For this review, take the finished solid that the model builds, in its own axes (mm). A direction names the side the tool comes from. Round coordinates to 2 decimals unless told otherwise and drop trailing zeros. Order: outer loops, then holes, each group sorted by start corner. A loop starts at its lowest first (then second) coordinate and runs counter-clockwise, first axis right, second up. Notation, with made-up numbers: (-39.75, 13) - (1.25, 13) arc R14 ccw to (1.25, 27) - close; hole circle Ø8 at (16.25, 3.5). An arc over 180 degrees is marked (long way). One line per question, with ' | ' between items.
```python
from build123d import *

# Parameters (mm, degrees)
BOSS_EXTRUDE1_DEPTH                               = 25
SKETCH2_W                                         = 18.5
SKETCH2_H                                         = 19
CUT_EXTRUDE1_DEPTH                                = 25
COUNTERBORE_FOR_PAN_HEAD_SCREW_OF_M61_D           = 6.6
COUNTERBORE_FOR_PAN_HEAD_SCREW_OF_M61_CBORE_D     = 13
COUNTERBORE_FOR_PAN_HEAD_SCREW_OF_M61_CBORE_DEPTH = 4.6
FILETE1_R                                         = 5
FILETE2_R                                         = 2


with BuildPart() as part:
    # Sketch1 → Boss-Extrude1 (new body)
    with BuildSketch(Plane(origin=(0, 0, 0), x_dir=(1, 0, 0), z_dir=(0, 1, 0))):
        Polygon((-52.5, 0), (52.5, 0), (65, -20), (65, -35), (45, -35), (45, -5), (-45, -5), (-45, -35), (-65, -35), (-65, -20), align=None)
    extrude(amount=BOSS_EXTRUDE1_DEPTH)

    # Sketch2 → Cut-Extrude1 (cut)
    with BuildSketch(Plane(origin=(0, 0, 0), x_dir=(-1, 0, 0), z_dir=(0, 0, -1))):
        with Locations((-58.75, 12.5)):
            Rectangle(SKETCH2_W, SKETCH2_H)
        with Locations((58.75, 12.5)):
            Rectangle(SKETCH2_W, SKETCH2_H)
    extrude(amount=-CUT_EXTRUDE1_DEPTH, mode=Mode.SUBTRACT)

    # Counterbore for pan head screw of M61 (through all)
    with Locations(Plane(origin=(0, 0, 25), x_dir=(-1, 0, 0), z_dir=(0, 0, -1))):
        with Locations((-57.25, 12.5), (57.25, 12.5)):
            CounterBoreHole(COUNTERBORE_FOR_PAN_HEAD_SCREW_OF_M61_D / 2, COUNTERBORE_FOR_PAN_HEAD_SCREW_OF_M61_CBORE_D / 2, COUNTERBORE_FOR_PAN_HEAD_SCREW_OF_M61_CBORE_DEPTH)

    # Filete1
    filete1_edges = [part.edges().sort_by_distance(p)[0] for p in [
        (-52.5, 23.5, 0),
        (52.5, 23.5, 0),
        (65, 23.5, 20),
        (-65, 23.5, 20),
        (52.5, 1.5, 0),
        (65, 1.5, 20),
        (-52.5, 1.5, 0),
        (-65, 1.5, 20),
    ]]
    fillet(filete1_edges, radius=FILETE1_R)

    # Filete2
    filete2_edges = [part.edges().sort_by_distance(p)[0] for p in [
        (45, 12.5, 5),
        (-45, 12.5, 5),
    ]]
    fillet(filete2_edges, radius=FILETE2_R)


solid = part.part
```
(1) Mouldability with a two-part tool opening along Y and no side actions: class faces 4 (the flat face through (-54, 14, 29.6)), 5 (the flat face through (59.03, 1.48, 10.45)) as released by +Y, released by -Y, zero draft, split by the parting line, or undercut.
Output values:
face 4: undercut | face 5: zero draft
(2) For faces 1 (the cylindrical face through (51.05, 14.45, 27.27)), 2 (the flat face through (56, 22, 15)), 3 (the flat face through (-55, 3, 15)), list the 3-axis set-ups (+Z, -Z, +X, -X, +Y, -Y) from which the entire face can be reached by the end or side of a thin tool; tool diameter is ignored.
Output values:
face 1: -Z | face 2: -Z, +X | face 3: -Z, -X
(3) For probe 1 along X at (y, z) = (10.5, 18); probe 2 along X at (y, z) = (12, 32); probe 3 along Y at (x, z) = (-57.25, 28.25), list the stretches that pass through material, from the lowest coordinate up. Write a range as [from, to].
Output values:
probe 1: [-49.5, -45], [45, 49.5] | probe 2: [-65, -60.51], [-53.99, -45], [45, 53.99], [60.51, 65] | probe 3: [0, 6], [19, 25]
(4) We need section A-A on z = 16. State the section outline as (x, y) points, plus the area to 3 significant figures.
Output values:
outline: (-62.5, 0) - (-45, 0) - (-45, 25) - (-62.5, 25) - (-62.5, 22) - (-49.5, 22) - (-49.5, 3) - (-62.5, 3) - close; (45, 0) - (62.5, 0) - (62.5, 3) - (49.5, 3) - (49.5, 22) - (62.5, 22) - (62.5, 25) - (45, 25) - close | area: 381 mm^2
(5) Insertion check: pin 1 (8 mm diameter, centred on x = 57, y = 12.5, fed in from -Z); pin 2 (4 mm diameter, centred on y = 21.5, z = 6.5, fed in from -X); pin 3 (6 mm diameter, centred on y = 21, z = 18, fed in from +X). Each pin has a flat end and moves straight along its axis. Give the tip position at first contact, or say it passes through.
Output values:
pin 1: z = 29.6 | pin 2: x = -57.77 | pin 3: x = 64.96
(6) We need section B-B on x = 57.25. State the section outline as (y, z) points, plus the area to 3 significant figures.
Output values:
outline: (0, 7.6) - (3, 7.6) - (3, 25) - (6, 25) - (6, 29.6) - (9.2, 29.6) - (9.2, 35) - (0, 35) - close; (15.8, 29.6) - (19, 29.6) - (19, 25) - (22, 25) - (22, 7.6) - (25, 7.6) - (25, 35) - (15.8, 35) - close | area: 259 mm^2
(7) We need section D-D on y = 23.5. State the section outline as (x, z) points.
Output values:
outline: (-65, 21.43) arc R5 ccw to (-64.24, 18.78) - (-53.97, 2.35) arc R5 ccw to (-49.73, 0) - (49.73, 0) arc R5 ccw to (53.97, 2.35) - (64.24, 18.78) arc R5 ccw to (65, 21.43) - (65, 35) - (45, 35) - (45, 7) arc R2 cw to (43, 5) - (-43, 5) arc R2 cw to (-45, 7) - (-45, 35) - (-65, 35) - close
(8) We need section C-C on y = 12.5. Give the number of separate pieces and of enclosed holes in the cut face, plus the area to 3 significant figures.
Output values:
separate pieces: 3 | enclosed holes: 0 | area: 886 mm^2
